```python
from build123d import *


with BuildPart() as part:
    # 草图1 → 旋转1 (revolve)
    with BuildSketch(Plane.XY, mode=Mode.PRIVATE) as revolve_1_sk:
        with BuildLine():
            Line((-44.2, 177), (-40.83502586, 177))
            ThreePointArc((-40.83502586, 177), (-40.152047165, 176.730438295), (-39.837278274, 176.067080205))
            Line((-39.837278274, 176.067080205), (-28, 0))
            Line((-28, 0), (0, 0))
            Line((0, 0), (0, -0.3))
            Line((0, -0.3), (-28.280507758, -0.3))
            Line((-28.280507758, -0.3), (-40.13660255, 176.046956143))
            ThreePointArc((-40.13660255, 176.046956143), (-40.356940774, 176.511306806), (-40.83502586, 176.7))
            Line((-40.83502586, 176.7), (-44.2, 176.7))
            Line((-44.2, 176.7), (-44.2, 175.4))
            Line((-44.2, 175.4), (-44.5, 175.4))
            Line((-44.5, 175.4), (-44.5, 176.7))
            ThreePointArc((-44.5, 176.7), (-44.412132034, 176.912132034), (-44.2, 177))
        make_face()
    revolve(revolve_1_sk.sketch.rotate(Axis((0, 0, 0), (0, -1, 0)), 270), axis=Axis((0, 0, 0), (0, -1, 0)))


solid = part.part
```
Part model, mm, in its own coordinate system. A direction names the side the tool comes from. Coordinates: 2 decimals unless noted, no trailing zeros. Loops run counter-clockwise (first coordinate to the right, second up) from the corner with the lowest first, then second, coordinate; pieces in that order, holes last. Notation, with made-up numbers: (88, 30) - (100, 30) arc R19 ccw to (100, 48) - close; hole circle Ø10 at (-25, 21.25). An arc over 180 degrees is marked (long way). Write item = value, one per line. Start each with the question number.
Item 1: 3-axis set-ups, long thin cutter, end or side, ignore diameter. For faces 5 (the cylindrical face through (43.15, 176.04, -9.58)), 6 (the flat face through (0, 0, 0)), 7 (the flat face through (39, 177, 13)): which of +Z, -Z, +X, -X, +Y, -Y reach the whole face in a straight line?
Item 2: Cut at C-C, the plane y = 78. Give the cut face in (x, z).
Item 3: Cut at B-B, the plane x = 0. Give the cut face in (y, z).
Item 4: Wall check: L1, parallel to X at y = 175.75, z = 0; L2, parallel to X at y = 176.25, z = 0; L3, parallel to Z at x = -15, y = 119. Give the ranges that are in metal, low to high. Write a range as from..to.
Item 5: Cut at A-A, the plane z = 0. Give the cut face in (x, y), and give its area (3 significant figures).
Item 6: Flat gauge pins, fed straight in: pin 1 Ø6 at (y, z) = (147.5, 18.5) entering from +X; pin 2 Ø1 at (y, z) = (35.5, -7) entering from -X; pin 3 Ø2 at (x, y) = (-30.5, 105) entering from -Z. Where does each tip first touch, or does it go through?
Item 7: Mould opens along Z. For faces 1 (the conical face through (-10.163, 86.801, 32.273)), 2 (the cylindrical face through (-30.075, 176.059, -32.798)), 3 (the flat face through (0, -0.3, 0)), 4 (the flat face through (13, 176.7, -39)) say: released by +Z, released by -Z, zero draft, split by the parting line, or undercut.
Item 8: Cut at D-D, the plane y = 97. Give the cut face in (x, z).
The answers:
q1.face_5 = -Y
q1.face_6 = +Y
q1.face_7 = +Z, -Z, +X, -X, +Y
q2.outline = circle Ø67.09 at (0, 0); hole circle Ø66.49 at (0, 0)
q3.outline = (-0.3, -28.28) - (176.05, -40.14) arc R0.7 cw to (176.7, -40.84) - (176.7, -44.2) - (175.4, -44.2) - (175.4, -44.5) - (176.7, -44.5) arc R0.3 ccw to (177, -44.2) - (177, -40.84) arc R1 ccw to (176.07, -39.84) - (0, -28) - (0, 28) - (176.07, 39.84) arc R1 ccw to (177, 40.84) - (177, 44.2) arc R0.3 ccw to (176.7, 44.5) - (175.4, 44.5) - (175.4, 44.2) - (176.7, 44.2) - (176.7, 40.84) arc R0.7 cw to (176.05, 40.14) - (-0.3, 28.28) - close
q4.L1 = -44.5..-44.2, -40.12..-39.82, 39.82..40.12, 44.2..44.5
q4.L2 = -44.5..-44.2, -40.18..-39.87, 39.87..40.18, 44.2..44.5
q4.L3 = -33.06..-32.73, 32.73..33.06
q5.outline = (-44.5, 175.4) - (-44.2, 175.4) - (-44.2, 176.7) - (-40.84, 176.7) arc R0.7 cw to (-40.14, 176.05) - (-28.28, -0.3) - (28.28, -0.3) - (40.14, 176.05) arc R0.7 cw to (40.84, 176.7) - (44.2, 176.7) - (44.2, 175.4) - (44.5, 175.4) - (44.5, 176.7) arc R0.3 ccw to (44.2, 177) - (40.84, 177) arc R1 ccw to (39.84, 176.07) - (28, 0) - (-28, 0) - (-39.84, 176.07) arc R1 ccw to (-40.84, 177) - (-44.2, 177) arc R0.3 ccw to (-44.5, 176.7) - close
q5.area = 127 mm2
q6.pin_1 = 34.95
q6.pin_2 = -30
q6.pin_3 = -19.5
q7.face_1 = undercut
q7.face_2 = split by the parting line
q7.face_3 = zero draft
q7.face_4 = undercut
q8.outline = circle Ø69.64 at (0, 0); hole circle Ø69.04 at (0, 0)
